Design review of the part built by this model. Coordinates are the model's own, in mm. Face numbers are marked on the shaded views. A direction names the side the tool comes from. Coordinates: 2 decimals unless noted, no trailing zeros. Write each loop counter-clockwise with the first axis right and the second up, starting at its lowest first coordinate (ties: lowest second). Pieces come first, ordered by that corner, then holes.
```python
from build123d import *

# Parameters (mm, degrees)
EXTRUDE_2_DEPTH               = 50
CUT_EXTRUDE_1_DEPTH           = 122.86057607
CUT_EXTRUDE_1_DEPTH_BACK      = 122.86057607
SKETCH_2_R                    = 8
CUT_EXTRUDE_8_DEPTH           = 85.409715081
CUT_EXTRUDE_8_DEPTH_BACK      = 85.409715081
SKETCH_3_W                    = 34.567648094
SKETCH_3_H                    = 27
SKETCH_3_W_2                  = 34.56764798
SKETCH_3_H_2                  = 5
CHAMFER_1_SIZE                = 5
HOLE_WIZARD_M10_1_D           = 11
HOLE_WIZARD_M10_1_CBORE_D     = 22
HOLE_WIZARD_M10_1_CBORE_DEPTH = 0.5


with BuildPart() as part:
    # 草图1 → 凸台-拉伸2 (new, symmetric)
    with BuildSketch(Plane.XY):
        with BuildLine():
            Line((-50, -10), (50, -10))
            Line((50, -10), (50, 10))
            Line((50, 10), (-35, 10))
            ThreePointArc((-35, 10), (-60.606601718, 20.606601718), (-50, -5))
            Line((-50, -5), (-50, -10))
        make_face()
    extrude(amount=EXTRUDE_2_DEPTH, both=True)

    # 草图2 → 切除-拉伸1 (cut, two sides: drawn at the far end of the back side and taken through both)
    with BuildSketch(Plane.XY.offset(50).offset(-CUT_EXTRUDE_1_DEPTH_BACK)):
        with Locations((-50, 10)):
            Circle(SKETCH_2_R)
    extrude(amount=CUT_EXTRUDE_1_DEPTH + CUT_EXTRUDE_1_DEPTH_BACK, mode=Mode.SUBTRACT)

    # 草图3 → 切除-拉伸8 (cut, two sides: drawn at the far end of the back side and taken through both)
    with BuildSketch(Plane(origin=(0, 10, 0), x_dir=(1, 0, 0), z_dir=(0, 1, 0)).offset(-CUT_EXTRUDE_8_DEPTH_BACK)):
        Polygon((-69.567648094, 22.997195123), (-35, 22.997195123), (-35, 50), (-69.107419327, 50), align=None)
        with Locations((-52.283824047, -9.502804877)):
            Rectangle(SKETCH_3_W, SKETCH_3_H)
        with Locations((-52.28382399, -47.5)):
            Rectangle(SKETCH_3_W_2, SKETCH_3_H_2)
    extrude(amount=CUT_EXTRUDE_8_DEPTH + CUT_EXTRUDE_8_DEPTH_BACK, mode=Mode.SUBTRACT)

    # 倒角1
    chamfer_1_edges = [part.edges().sort_by_distance(p)[0] for p in [
        (50, 10, 0),
    ]]
    chamfer(chamfer_1_edges, length=CHAMFER_1_SIZE)

    # M10 六角头螺栓的柱形沉头孔1 (through all)
    with Locations(Plane(origin=(5, 10, -30), x_dir=(0, 0, 1), z_dir=(0, 1, 0))):
        with Locations((0, 0)):
            hole_wizard_m10_1 = CounterBoreHole(HOLE_WIZARD_M10_1_D / 2, HOLE_WIZARD_M10_1_CBORE_D / 2, HOLE_WIZARD_M10_1_CBORE_DEPTH)

    # 镜向1: M10 六角头螺栓的柱形沉头孔1 across plane
    add(hole_wizard_m10_1.mirror(Plane.XY), mode=Mode.SUBTRACT)


solid = part.part
```
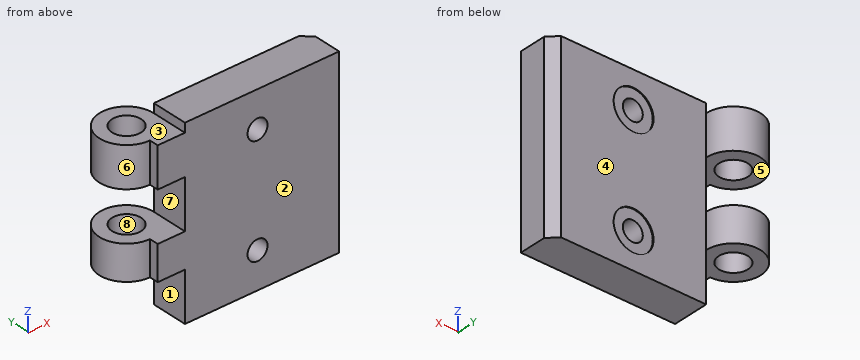
(1) Consider section C-C (z = -7). Give the boundary of the cut face in (x, y), plus the area to 3 significant figures.
(2) Wall thickness on line 1 (X direction, y = -6.5, z = 6); line 2 (Y direction, x = -25, z = -31.5); line 3 (X direction, y = -8, z = -15): over which ranges is each line inside the solid? List them lowest first.
(3) Insertion check: pin 1 Ø6 at (y, z) = (1.5, -43) entering from -X; pin 2 Ø15 at (x, y) = (-49, 15) entering from +Z; pin 3 Ø13 at (x, y) = (-50, 10) entering from -Z; pin 4 Ø1.5 at (y, z) = (-7.5, 28.5) entering from -X. Each pin has a flat end and moves straight along its axis. Give the tip position at first contact, or say it passes through.
(4) For the marked faces 1, 2, 3, 4 and 5, list the 3-axis set-ups (+Z, -Z, +X, -X, +Y, -Y) from which the entire face can be reached by the end or side of a thin tool; tool diameter is ignored.
(5) Consider section D-D (y = 13.5). Give the boundary of the cut face in (x, z).
(6) Consider section B-B (z = -30). Give the boundary of the cut face in (x, y).
(7) Consider section A-A (z = 30). Give the boundary of the cut face in (x, y), plus the area to 3 significant figures.
(8) Mouldability with a two-part tool opening along X and no side actions: class the marked faces 6, 7 and 8 as +X half, -X half, draft (parallel to the pull), parting line (faces both ways), or undercut.
Results:
1. outline: (-50, -10) - (50, -10) - (50, 5) - (45, 10) - (-35, 10) arc R15 ccw (long way) to (-50, -5) - close; hole circle Ø16 at (-50, 10)
1. area: 2,320 mm2
2. line 1: x = -35 to 50
2. line 2: y = -10 to 10
2. line 3: x = -50 to 50
3. pin 1: stops at x = -35
3. pin 2: stops at z = 45
3. pin 3: passes through
3. pin 4: stops at x = -50
4. face 1: -Z, -X, +Y, -Y
4. face 2: +Z, -Z, +X, -X, -Y
4. face 3: +Z, -X, +Y, -Y
4. face 4: +Z, -Z, +X, +Y
4. face 5: -X, +Y, -Y
5. outline: (-64.59, -23) - (-57.19, -23) - (-57.19, -4) - (-64.59, -4) - close; (-64.59, 23) - (-57.19, 23) - (-57.19, 45) - (-64.59, 45) - close; (-42.81, -23) - (-35.41, -23) - (-35.41, -4) - (-42.81, -4) - close; (-42.81, 23) - (-35.41, 23) - (-35.41, 45) - (-42.81, 45) - close
6. outline: (-35, -10) - (-0.5, -10) - (-0.5, 9.5) - (-6, 9.5) - (-6, 10) - (-35, 10) - close; (10.5, -10) - (50, -10) - (50, 5) - (45, 10) - (16, 10) - (16, 9.5) - (10.5, 9.5) - close
7. outline: (-50, -10) - (-0.5, -10) - (-0.5, 9.5) - (-6, 9.5) - (-6, 10) - (-35, 10) arc R15 ccw (long way) to (-50, -5) - close; (10.5, -10) - (50, -10) - (50, 5) - (45, 10) - (16, 10) - (16, 9.5) - (10.5, 9.5) - close; hole circle Ø16 at (-50, 10)
7. area: 2,090 mm2
8. face 6: parting line
8. face 7: -X half
8. face 8: undercut
